```python
from build123d import *

# Parameters (mm, degrees)
SKETCH1_R           = 15
BOSS_EXTRUDE1_DEPTH = 10
SKETCH2_W           = 100
SKETCH2_H           = 110
BOSS_EXTRUDE2_DEPTH = 10
CHAMFER1_SIZE       = 2


with BuildPart() as part:
    # Sketch1 → Boss-Extrude1 (new body)
    with BuildSketch(Plane.XY):
        with BuildLine():
            Line((139, -40), (139, -85))
            Line((139, -85), (99, -85))
            Line((99, -85), (99, -40))
            ThreePointArc((99, -40), (119, -20), (139, -40))
        make_face()
        with Locations((119, -40)):
            Circle(SKETCH1_R, mode=Mode.SUBTRACT)
    extrude(amount=-BOSS_EXTRUDE1_DEPTH)

    # Sketch2 → Boss-Extrude2 (add)
    with BuildSketch(Plane.XZ.offset(85)):
        with Locations((119, -15)):
            Rectangle(SKETCH2_W, SKETCH2_H)
    extrude(amount=BOSS_EXTRUDE2_DEPTH)

    # Chamfer1
    chamfer1_edges = [part.edges().sort_by_distance(p)[0] for p in [
        (169, -95, -15),
        (119, -95, 40),
        (69, -95, -15),
        (119, -95, -70),
    ]]
    chamfer(chamfer1_edges, length=CHAMFER1_SIZE)


solid = part.part
```
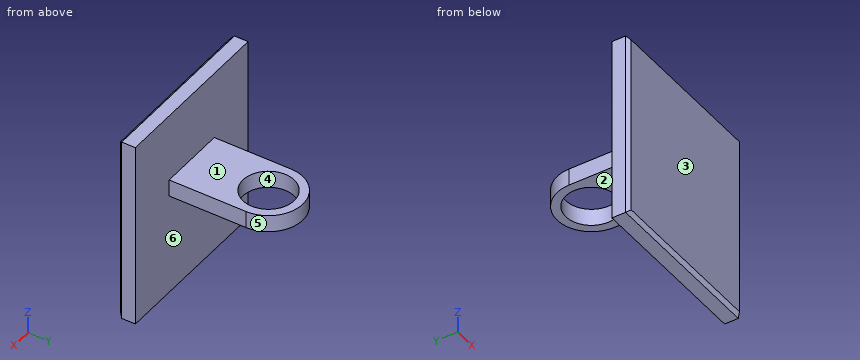
Part model, mm, in its own coordinate system. Face numbers are marked on the shaded views. A direction names the side the tool comes from. Round coordinates to 2 decimals unless told otherwise and drop trailing zeros. Order: outer loops, then holes, each group sorted by start corner. A loop starts at its lowest first (then second) coordinate and runs counter-clockwise, first axis right, second up. Notation, with made-up numbers: M 29,27 L 55,27 A28 ccw 55,62 Z; hole C 65.5,83 d9. An arc over 180 degrees is marked long. Answer in a Markdown table with one row per item. Add a question column.
Q1. Cut at B-B on z = -7. Give the cut face in (x, y), and give its area (3 significant figures).
Q2. Mould opens along X. For the marked faces 4, 5 and 6 say: +X half, -X half, draft (parallel to the pull), parting line (faces both ways), or undercut.
Q3. Cut at C-C on y = -42. Give the cut face in (x, z).
Q4. Cut at A-A on x = 119. Give the cut face in (y, z), and give its area (3 significant figures).
Q5. Cut at D-D on y = -82. Give the cut face in (x, z), and give its area (3 significant figures).
Q6. 3-axis set-ups, long thin cutter, end or side, ignore diameter. For the marked faces 1, 2 and 3: which of +Z, -Z, +X, -X, +Y, -Y reach the whole face in a straight line?
Q7. Wall check: L1, parallel to Z at x = 121.5, y = -73; L2, parallel to Y at x = 119, z = -7.5; L3, parallel to Y at x = 105.5, z = -36. Give the ranges that are in metal, low to high. Write a range as from..to.
Q8. Pin check, flat tips, straight feed: pin 1 (11 mm diameter, centred on y = -71.5, z = -3.5, fed in from -X); pin 2 (12 mm diameter, centred on x = 82, y = -79.5, fed in from -Z); pin 3 (8 mm diameter, centred on y = -59.5, z = -7, fed in from +X); pin 4 (4 mm diameter, centred on y = -29.5, z = -2.5, fed in from +X). Stop position of each tip, or through.
Established:
| question | item | result |
|---|---|---|
| 1 | outline | M 69,-93 L 71,-95 L 167,-95 L 169,-93 L 169,-85 L 139,-85 L 139,-40 A20 ccw 99,-40 L 99,-85 L 69,-85 Z; hole C 119,-40 d30 |
| 1 | area | 2,720 mm2 |
| 2 | face 4 | undercut |
| 2 | face 5 | parting line |
| 2 | face 6 | draft |
| 3 | outline | M 99,-10 L 104.13,-10 L 104.13,0 L 99,0 Z; M 133.87,-10 L 139,-10 L 139,0 L 133.87,0 Z |
| 4 | outline | M -95,-68 L -93,-70 L -85,-70 L -85,-10 L -55,-10 L -55,0 L -85,0 L -85,40 L -93,40 L -95,38 Z; M -25,-10 L -20,-10 L -20,0 L -25,0 Z |
| 4 | area | 1,450 mm2 |
| 5 | outline | M 99,-10 L 139,-10 L 139,0 L 99,0 Z |
| 5 | area | 400 mm2 |
| 6 | face 1 | +Z, +X, -X, +Y |
| 6 | face 2 | -Z, +X, -X, +Y |
| 6 | face 3 | +Z, -Z, +X, -X, -Y |
| 7 | L1 | z = -10..0 |
| 7 | L2 | y = -95..-55, -25..-20 |
| 7 | L3 | y = -95..-85 |
| 8 | pin 1 | stops at x = 99 |
| 8 | pin 2 | stops at z = -70 |
| 8 | pin 3 | stops at x = 139 |
| 8 | pin 4 | stops at x = 137.1 |
